Check sheet for the modelled part. Datum: model origin and axes. Units: mm. A direction names the side the tool comes from. Coordinates: 2 decimals unless noted, no trailing zeros. Write each loop counter-clockwise with the first axis right and the second up, starting at its lowest first coordinate (ties: lowest second). Pieces come first, ordered by that corner, then holes. Notation, with made-up numbers: (-18, 3.25) -> (28, 3.25) arc R8 cw to (28, 10.25) -> close; hole circle Ø10 at (5.5, -29). An arc over 180 degrees is marked (long way). Put each result on its own line as item: value.
```python
from build123d import *

# Parameters (mm, degrees)
BOSS_EXTRUDE1_DEPTH            = 20
CUT_EXTRUDE1_DEPTH             = 10
CHAMFER1_SIZE                  = 1
FILLET1_R                      = 1.5
FILLET2_R                      = 0.5
F_2_2_2_2_DIAMETER_HOLE1_D     = 2.2
F_2_2_2_2_DIAMETER_HOLE1_DEPTH = 5
F_2_2_2_2_DIAMETER_HOLE1_TIP   = 0.660946681


with BuildPart() as part:
    # Sketch1 → Boss-Extrude1 (new body)
    with BuildSketch(Plane(origin=(0, 0, 0), x_dir=(1, 0, 0), z_dir=(0, 1, 0))):
        Polygon((0, 0), (16.5, 0), (16.5, 4), (30, 4), (30, 5), (15.5, 5), (15.5, 1), (0, 1), align=None)
    extrude(amount=BOSS_EXTRUDE1_DEPTH)

    # Sketch2 → Cut-Extrude1 (cut)
    with BuildSketch(Plane(origin=(0, 0, -5), x_dir=(-1, 0, 0), z_dir=(0, 0, -1))):
        with BuildLine():
            Line((-10.5, 16), (-10.5, 4))
            ThreePointArc((-10.5, 4), (-11.75, 2.75), (-13, 4))
            Line((-13, 4), (-13, 16))
            ThreePointArc((-13, 16), (-11.75, 17.25), (-10.5, 16))
        make_face()
        with BuildLine():
            Line((-5, 16), (-5, 4))
            ThreePointArc((-5, 4), (-3.75, 2.75), (-2.5, 4))
            Line((-2.5, 4), (-2.5, 16))
            ThreePointArc((-2.5, 16), (-3.75, 17.25), (-5, 16))
        make_face()
    extrude(amount=-CUT_EXTRUDE1_DEPTH, mode=Mode.SUBTRACT)

    # Chamfer1
    chamfer1_edges = [part.edges().sort_by_distance(p)[0] for p in [
        (0, 0, -0.5),
        (30, 20, -4.5),
        (0, 20, -0.5),
        (30, 0, -4.5),
    ]]
    chamfer(chamfer1_edges, length=CHAMFER1_SIZE)

    # Fillet1
    fillet1_edges = [part.edges().sort_by_distance(p)[0] for p in [
        (15.5, 10, -5),
        (16.5, 10, 0),
    ]]
    fillet(fillet1_edges, radius=FILLET1_R)

    # Fillet2
    fillet2_edges = [part.edges().sort_by_distance(p)[0] for p in [
        (15.5, 10, -1),
        (16.5, 10, -4),
    ]]
    fillet(fillet2_edges, radius=FILLET2_R)

    # Ø2.2 (2.2) Diameter Hole1
    with Locations(Plane.XY.offset(-4)):
        with Locations((27.25, 16.75), (27.25, 5.75)):
            Hole(F_2_2_2_2_DIAMETER_HOLE1_D / 2, depth=F_2_2_2_2_DIAMETER_HOLE1_DEPTH)
            with Locations((0, 0, -(F_2_2_2_2_DIAMETER_HOLE1_DEPTH + F_2_2_2_2_DIAMETER_HOLE1_TIP / 2))):  # 118° drill point
                Cone(0, F_2_2_2_2_DIAMETER_HOLE1_D / 2, F_2_2_2_2_DIAMETER_HOLE1_TIP, mode=Mode.SUBTRACT)


solid = part.part
```
Q1. Cross-section at A-A (x = 27.25). Record the cut outline in (y, z).
Recorded:
outline: (0, -5) -> (4.65, -5) -> (4.65, -4) -> (0, -4) -> close; (6.85, -5) -> (15.65, -5) -> (15.65, -4) -> (6.85, -4) -> close; (17.85, -5) -> (20, -5) -> (20, -4) -> (17.85, -4) -> close
Q2. Cross-section at D-D (y = 11.25). Record the cut outline in (x, z).
Recorded:
outline: (0, -1) -> (2.5, -1) -> (2.5, 0) -> (0, 0) -> close; (5, -1) -> (10.5, -1) -> (10.5, 0) -> (5, 0) -> close; (13, -1) -> (15, -1) arc R0.5 cw to (15.5, -1.5) -> (15.5, -3.5) arc R1.5 ccw to (17, -5) -> (30, -5) -> (30, -4) -> (17, -4) arc R0.5 cw to (16.5, -3.5) -> (16.5, -1.5) arc R1.5 ccw to (15, 0) -> (13, 0) -> close
Q3. Material ranges on line 1 along Y through (x, z) = (27.25, -4.8); line 2 along Z through (x, y) = (6.75, 16.75); line 3 along X through (y, z) = (3.25, -1.75), recorded low to high.
Recorded:
line 1: y = 0 to 4.65, 6.85 to 15.65, 17.85 to 20
line 2: z = -1 to 0
line 3: x = 15.5 to 16.5
Q4. Tool access check on faces 4 (the flat face through (8, 10, -1)), 5 (the flat face through (29.5, 0.5, -4.5)), 6 (the flat face through (16.5, 10, -2)), 7 (the cylindrical face through (3.72, 17.25, -0.51)). Record the directions out of +Z, -Z, +X, -X, +Y, -Y that give a thin tool (end or side, any length) a straight path to the whole face; none if there is none.
Recorded:
face 4: -Z, -X, +Y, -Y
face 5: +Z, -Z, +X, -Y
face 6: +Z, +X, +Y, -Y
face 7: +Z, -Z
Q5. Depth check by flat-ended pin: P1, Ø2, axis at y = 14.5, z = -2.5, coming from the -X side; P2, Ø1.1, axis at y = 7.5, z = -0.5, coming from the +X side; P3, Ø8, axis at x = 12.5, y = 9.5, coming from the -Z side. Enter the tip coordinate at first touch or a pass-through.
Recorded:
P1: stops at x = 15.5
P2: stops at x = 16.43
P3: stops at z = -4.91
Q6. Cross-section at C-C (x = 3.75). Record the cut outline in (y, z), plus the area to 3 significant figures.
Recorded:
outline: (0, -1) -> (2.75, -1) -> (2.75, 0) -> (0, 0) -> close; (17.25, -1) -> (20, -1) -> (20, 0) -> (17.25, 0) -> close
area: 5.50 mm2
Q7. Cross-section at B-B (y = 16.75). Record the cut outline in (x, z), plus the area to 3 significant figures.
Recorded:
outline: (0, -1) -> (2.75, -1) -> (2.75, 0) -> (0, 0) -> close; (4.75, -1) -> (10.75, -1) -> (10.75, 0) -> (4.75, 0) -> close; (12.75, -1) -> (15, -1) arc R0.5 cw to (15.5, -1.5) -> (15.5, -3.5) arc R1.5 ccw to (17, -5) -> (26.15, -5) -> (26.15, -4) -> (17, -4) arc R0.5 cw to (16.5, -3.5) -> (16.5, -1.5) arc R1.5 ccw to (15, 0) -> (12.75, 0) -> close; (28.35, -5) -> (30, -5) -> (30, -4) -> (28.35, -4) -> close
area: 26.9 mm2
Q8. Mould release check, pull along Y, two halves, no side actions. Record for faces 1 (the cylindrical face through (11.72, 2.75, -0.51)), 2 (the flat face through (29.5, 19.5, -4.5)), 3 (the flat face through (23, 10, -4)): released by +Y, released by -Y, zero draft, split by the parting line, or undercut.
Recorded:
face 1: undercut
face 2: released by +Y
face 3: zero draft
